from build123d import *

# Parameters (mm, degrees)
PROFILE_SECTION_35X35_R     = 2.625
PROFILE_EXTRUSION_L15_DEPTH = 7.5


with BuildPart() as part:
    # Profile Section 35x35 → Profile Extrusion L15 (new, symmetric)
    with BuildSketch(Plane.XY):
        with BuildLine():
            Line((-13.8, -17.5), (-6, -17.5))
            ThreePointArc((-6, -17.5), (-5, -16.5), (-6, -15.5))
            Line((-6, -15.5), (-10.1, -15.5))
            Line((-10.1, -15.5), (-10.1, -11.3))
            Line((-10.1, -11.3), (-6, -9))
            Line((-6, -9), (0, -9))
            Line((0, -9), (6, -9))
            Line((6, -9), (10.1, -11.3))
            Line((10.1, -11.3), (10.1, -15.5))
            Line((10.1, -15.5), (6, -15.5))
            ThreePointArc((6, -15.5), (5, -16.5), (6, -17.5))
            Line((6, -17.5), (13.8, -17.5))
            Line((13.8, -17.5), (15.5, -17.5))
            ThreePointArc((15.5, -17.5), (16.914213562, -16.914213562), (17.5, -15.5))
            Line((17.5, -15.5), (17.5, -6))
            ThreePointArc((17.5, -6), (16.5, -5), (15.5, -6))
            Line((15.5, -6), (15.5, -10.1))
            Line((15.5, -10.1), (11.3, -10.1))
            Line((11.3, -10.1), (9, -6))
            Line((9, -6), (9, 0))
            Line((9, 0), (9, 6))
            Line((9, 6), (11.3, 10.1))
            Line((11.3, 10.1), (15.5, 10.1))
            Line((15.5, 10.1), (15.5, 6))
            ThreePointArc((15.5, 6), (16.5, 5), (17.5, 6))
            Line((17.5, 6), (17.5, 15.5))
            ThreePointArc((17.5, 15.5), (16.914213562, 16.914213562), (15.5, 17.5))
            Line((15.5, 17.5), (13.8, 17.5))
            Line((13.8, 17.5), (6, 17.5))
            ThreePointArc((6, 17.5), (5, 16.5), (6, 15.5))
            Line((6, 15.5), (10.1, 15.5))
            Line((10.1, 15.5), (10.1, 11.3))
            Line((10.1, 11.3), (6, 9))
            Line((6, 9), (0, 9))
            Line((0, 9), (-6, 9))
            Line((-6, 9), (-10.1, 11.3))
            Line((-10.1, 11.3), (-10.1, 15.5))
            Line((-10.1, 15.5), (-6, 15.5))
            ThreePointArc((-6, 15.5), (-5, 16.5), (-6, 17.5))
            Line((-6, 17.5), (-13.8, 17.5))
            Line((-13.8, 17.5), (-15.5, 17.5))
            ThreePointArc((-15.5, 17.5), (-16.914213562, 16.914213562), (-17.5, 15.5))
            Line((-17.5, 15.5), (-17.5, 6))
            ThreePointArc((-17.5, 6), (-16.5, 5), (-15.5, 6))
            Line((-15.5, 6), (-15.5, 8.244179001))
            Line((-15.5, 8.244179001), (-11.3, 8.244179001))
            Line((-11.3, 8.244179001), (-9, 6))
            Line((-9, 6), (-9, 0))
            Line((-9, 0), (-9, -6))
            Line((-9, -6), (-11.3, -10.1))
            Line((-11.3, -10.1), (-15.5, -10.1))
            Line((-15.5, -10.1), (-15.5, -6))
            ThreePointArc((-15.5, -6), (-16.5, -5), (-17.5, -6))
            Line((-17.5, -6), (-17.5, -15.5))
            ThreePointArc((-17.5, -15.5), (-16.914213562, -16.914213562), (-15.5, -17.5))
            Line((-15.5, -17.5), (-13.8, -17.5))
        make_face()
        with Locations((-13.8, -13.8)):
            Circle(PROFILE_SECTION_35X35_R, mode=Mode.SUBTRACT)
        with Locations((13.8, -13.8)):
            Circle(PROFILE_SECTION_35X35_R, mode=Mode.SUBTRACT)
        with Locations((-13.8, 11.944179001)):
            Circle(PROFILE_SECTION_35X35_R, mode=Mode.SUBTRACT)
        with BuildLine():
            Line((5.645056013, 4.937949232), (5.290657805, 4.583551024))
            ThreePointArc((5.290657805, 4.583551024), (6.999999998, -0.000156062), (5.290453424, -4.583786925))
            Line((5.290453424, -4.583786925), (5.650606112, -4.931597162))
            ThreePointArc((5.650606112, -4.931597162), (5.30628231, -5.300317731), (4.937949232, -5.645056013))
            Line((4.937949232, -5.645056013), (4.583551024, -5.290657805))
            ThreePointArc((4.583551024, -5.290657805), (0, -7), (-4.583551024, -5.290657805))
            Line((-4.583551024, -5.290657805), (-4.937949232, -5.645056013))
            ThreePointArc((-4.937949232, -5.645056013), (-5.303300859, -5.303300859), (-5.645056013, -4.937949232))
            Line((-5.645056013, -4.937949232), (-5.290657805, -4.583551024))
            ThreePointArc((-5.290657805, -4.583551024), (-6.996859079, -0.209673625), (-5.555626638, 4.258522357))
            Line((-5.555626638, 4.258522357), (-5.952457112, 4.562702525))
            ThreePointArc((-5.952457112, 4.562702525), (-5.64166709, 4.941820762), (-5.306773753, 5.299825689))
            Line((-5.306773753, 5.299825689), (-4.952988836, 4.946503977))
            ThreePointArc((-4.952988836, 4.946503977), (-0.252451062, 6.995446266), (4.583551024, 5.290657805))
            Line((4.583551024, 5.290657805), (4.937949232, 5.645056013))
            ThreePointArc((4.937949232, 5.645056013), (5.303300859, 5.303300859), (5.645056013, 4.937949232))
        make_face(mode=Mode.SUBTRACT)
        with Locations((13.8, 13.8)):
            Circle(PROFILE_SECTION_35X35_R, mode=Mode.SUBTRACT)
    extrude(amount=PROFILE_EXTRUSION_L15_DEPTH, both=True)


solid = part.part
Geometry check sheet. Reference: the model listing, model coordinates, mm. A direction names the side the tool comes from. Round coordinates to 2 decimals unless told otherwise and drop trailing zeros. Order: outer loops, then holes, each group sorted by start corner. A loop starts at its lowest first (then second) coordinate and runs counter-clockwise, first axis right, second up. Notation, with made-up numbers: (-22.5, 49) -> (-6.5, 49) arc R25 ccw to (-6.5, 66) -> close; hole circle Ø3 at (9.5, 59.25). An arc over 180 degrees is marked (long way). Use one line per item in the form item = value.
1. Scan lines: line 1 along Y through (x, z) = (-13.8, -2.5) (3 decimals); line 2 along Y through (x, z) = (13.8, -2.25) (3 decimals); line 3 along X through (y, z) = (-7.5, 3). Record each from-to range of solid material in increasing order. Write a range as from..to.
Working result:
line_1 = -17.5..-16.425, -11.175..-10.1, 8.244..9.319, 14.569..17.5
line_2 = -17.5..-16.425, -11.175..-10.1, 10.1..11.175, 16.425..17.5
line_3 = -17.5..-15.5, -9.84..9.84, 15.5..17.5
2. Cross-section at C-C, the plane x = 3. Enter the section's corners in (y, z), plus the area to 3 significant figures.
Working result:
outline = (-9, -7.5) -> (-6.32, -7.5) -> (-6.32, 7.5) -> (-9, 7.5) -> close; (6.32, -7.5) -> (9, -7.5) -> (9, 7.5) -> (6.32, 7.5) -> close
area = 80.3 mm^2
3. Set-up check for faces 5 (the face through (-7, 3, 7.5)), 6 (the face through (15.5, 8, 0)): record each of +Z, -Z, +X, -X, +Y, -Y from which the full face is reachable in a straight line by a thin tool's end or side.
Working result:
face_5 = +Z, +X, -X, +Y, -Y
face_6 = +Z, -Z
4. Cross-section at D-D, the plane y = 7.5. Enter the section's corners in (x, z), plus the area to 3 significant figures.
Working result:
outline = (-17.5, -7.5) -> (-15.5, -7.5) -> (-15.5, 7.5) -> (-17.5, 7.5) -> close; (-10.54, -7.5) -> (9.84, -7.5) -> (9.84, 7.5) -> (-10.54, 7.5) -> close; (15.5, -7.5) -> (17.5, -7.5) -> (17.5, 7.5) -> (15.5, 7.5) -> close
area = 366 mm^2
5. Cross-section at A-A, the plane y = 0. Enter the section's corners in (x, z).
Working result:
outline = (-9, -7.5) -> (-7, -7.5) -> (-7, 7.5) -> (-9, 7.5) -> close; (7, -7.5) -> (9, -7.5) -> (9, 7.5) -> (7, 7.5) -> close
6. Go/stop test with flat-tipped pins: pin 1 (2 mm diameter, centred on x = 5, y = 9.5, fed in from +Z); pin 2 (4 mm diameter, centred on y = -1.5, z = 4, fed in from +X). Record where each tip stops, or that it passes through.
Working result:
pin_1 = 7.5
pin_2 = 9
7. Cross-section at B-B, the plane y = -13. Enter the section's corners in (x, z), plus the area to 3 significant figures.
Working result:
outline = (-17.5, -7.5) -> (-16.3, -7.5) -> (-16.3, 7.5) -> (-17.5, 7.5) -> close; (-11.3, -7.5) -> (-10.1, -7.5) -> (-10.1, 7.5) -> (-11.3, 7.5) -> close; (10.1, -7.5) -> (11.3, -7.5) -> (11.3, 7.5) -> (10.1, 7.5) -> close; (16.3, -7.5) -> (17.5, -7.5) -> (17.5, 7.5) -> (16.3, 7.5) -> close
area = 72.0 mm^2
8. Mould release check, pull along X, two halves, no side actions. Record for faces 1 (the face through (13, -10.1, 0)), 2 (the face through (16.9, -16.93, 0.11)), 3 (the face through (-7, 3, -7.5)), 4 (the face through (-16.93, -16.9, 0.11)): pulls with the +X half, pulls with the -X half, needs draft (parallel to the pull), parting line crosses it, or undercut.
Working result:
face_1 = undercut
face_2 = pulls with the +X half
face_3 = needs draft
face_4 = pulls with the -X half
